from build123d import *

# Parameters (mm, degrees)
SKETCH1_W                                            = 152
SKETCH1_H                                            = 270
BOSS_EXTRUDE1_DEPTH                                  = 6
SKETCH2_R                                            = 35
CUT_EXTRUDE1_DEPTH                                   = 156.38661461
SKETCH5_R                                            = 6
SKETCH5_R_2                                          = 8.05
CUT_EXTRUDE2_DEPTH                                   = 5
SKETCH6_W                                            = 45
SKETCH6_H                                            = 70
CUT_EXTRUDE3_DEPTH                                   = 156.38661461
SKETCH7_W                                            = 45
SKETCH7_H                                            = 90
CUT_EXTRUDE4_DEPTH                                   = 156.38661461
SKETCH8_R                                            = 7.5
CUT_EXTRUDE5_DEPTH                                   = 2
SKETCH9_W                                            = 45
SKETCH9_H                                            = 65
CUT_EXTRUDE6_DEPTH                                   = 156.38661461
FILLET1_R                                            = 5
HOLE_SIZE_PER_SOCKET_HEAD_CAP_SCREW_TYPE_D           = 6.6
HOLE_SIZE_PER_SOCKET_HEAD_CAP_SCREW_TYPE_CBORE_D     = 11
HOLE_SIZE_PER_SOCKET_HEAD_CAP_SCREW_TYPE_CBORE_DEPTH = 6
HOLE_WIZARD_2_D                                      = 4.5
HOLE_WIZARD_2_CBORE_D                                = 8
HOLE_WIZARD_2_CBORE_DEPTH                            = 4
M8_CLEARANCE_HOLE1_D                                 = 8.4
CHAMFER1_SIZE                                        = 0.5


with BuildPart() as part:
    # Sketch1 → Boss-Extrude1 (new, symmetric)
    with BuildSketch(Plane(origin=(0, 0, 0), x_dir=(1, 0, 0), z_dir=(0, 1, 0))):
        Rectangle(SKETCH1_W, SKETCH1_H)
    extrude(amount=BOSS_EXTRUDE1_DEPTH, both=True)

    # Sketch2 → Cut-Extrude1 (cut, through all)
    with BuildSketch(Plane(origin=(0, 6, 0), x_dir=(1, 0, 0), z_dir=(0, 1, 0))):
        with Locations(Location((0, 0, 0), (0, 0, 270))):
            Circle(SKETCH2_R)
    extrude(amount=-CUT_EXTRUDE1_DEPTH, mode=Mode.SUBTRACT)

    # Sketch5 → Cut-Extrude2 (cut)
    with BuildSketch(Plane(origin=(0, 6, 0), x_dir=(1, 0, 0), z_dir=(0, 1, 0))):
        with Locations(Location((62.5, 62, 0), (0, 0, 270))):
            Circle(SKETCH5_R)
        with Locations(Location((-62.5, -62, 0), (0, 0, 270))):
            Circle(SKETCH5_R)
        with Locations(Location((62.5, 26, 0), (0, 0, 270))):
            Circle(SKETCH5_R_2)
        with Locations(Location((-62.5, 26, 0), (0, 0, 90))):
            Circle(SKETCH5_R_2)
        with Locations(Location((-62.5, -26, 0), (0, 0, 270))):
            Circle(SKETCH5_R_2)
        with Locations(Location((62.5, -26, 0), (0, 0, 90))):
            Circle(SKETCH5_R_2)
    extrude(amount=-CUT_EXTRUDE2_DEPTH, mode=Mode.SUBTRACT)

    # Sketch6 → Cut-Extrude3 (cut, through all)
    with BuildSketch(Plane(origin=(0, 6, 0), x_dir=(1, 0, 0), z_dir=(0, 1, 0))):
        Rectangle(SKETCH6_W, SKETCH6_H)
    extrude(amount=-CUT_EXTRUDE3_DEPTH, mode=Mode.SUBTRACT)

    # Sketch7 → Cut-Extrude4 (cut, through all)
    with BuildSketch(Plane(origin=(0, 6, 0), x_dir=(1, 0, 0), z_dir=(0, 1, 0))):
        with Locations((-53.5, 90)):
            Rectangle(SKETCH7_W, SKETCH7_H)
        with Locations((53.5, -90)):
            Rectangle(SKETCH7_W, SKETCH7_H)
    extrude(amount=-CUT_EXTRUDE4_DEPTH, mode=Mode.SUBTRACT)

    # Sketch8 → Cut-Extrude5 (cut)
    with BuildSketch(Plane.XZ.offset(6)):
        with Locations(Location((-20, 125, 0), (0, 0, 270))):
            Circle(SKETCH8_R)
        with Locations(Location((20, 125, 0), (0, 0, 90))):
            Circle(SKETCH8_R)
        with Locations(Location((20, -125, 0), (0, 0, 270))):
            Circle(SKETCH8_R)
        with Locations(Location((-20, -125, 0), (0, 0, 90))):
            Circle(SKETCH8_R)
    extrude(amount=-CUT_EXTRUDE5_DEPTH, mode=Mode.SUBTRACT)

    # Sketch9 → Cut-Extrude6 (cut, through all)
    with BuildSketch(Plane.XZ.offset(6)):
        with Locations((-53.5, 102.5)):
            Rectangle(SKETCH9_W, SKETCH9_H)
        with Locations((53.5, -102.5)):
            Rectangle(SKETCH9_W, SKETCH9_H)
    extrude(amount=-CUT_EXTRUDE6_DEPTH, mode=Mode.SUBTRACT)

    # Fillet1
    fillet1_edges = [part.edges().sort_by_distance(p)[0] for p in [
        (-31, 0, 70),
        (31, 0, -70),
        (22.5, 0, -35),
        (22.5, 0, 35),
        (-22.5, 0, 35),
        (-22.5, 0, -35),
        (-31, 0, -45),
        (31, 0, 45),
    ]]
    fillet(fillet1_edges, radius=FILLET1_R)

    # Hole size per socket head cap screw type 2 (through all)
    with Locations(Plane(origin=(0, 6, 0), x_dir=(1, 0, 0), z_dir=(0, 1, 0))):
        with Locations((-20, 125), (20, 125), (-20, -125), (20, -125)):
            CounterBoreHole(HOLE_SIZE_PER_SOCKET_HEAD_CAP_SCREW_TYPE_D / 2, HOLE_SIZE_PER_SOCKET_HEAD_CAP_SCREW_TYPE_CBORE_D / 2, HOLE_SIZE_PER_SOCKET_HEAD_CAP_SCREW_TYPE_CBORE_DEPTH)

    # 打孔尺寸(%根据)内六角圆柱头螺钉的类型2 (through all)
    with Locations(Plane(origin=(0, -6, 0), x_dir=(-1, 0, 0), z_dir=(0, -1, 0))):
        with Locations((62.5, -62), (-62.5, 62)):
            CounterBoreHole(HOLE_WIZARD_2_D / 2, HOLE_WIZARD_2_CBORE_D / 2, HOLE_WIZARD_2_CBORE_DEPTH)

    # M8 Clearance Hole1 (through all)
    with Locations(Plane(origin=(0, -6, 0), x_dir=(-1, 0, 0), z_dir=(0, -1, 0))):
        with Locations((62.5, -26), (62.5, 26), (-62.5, -26), (-62.5, 26)):
            Hole(M8_CLEARANCE_HOLE1_D / 2)

    # Chamfer1
    chamfer1_edges = [part.edges().sort_by_distance(p)[0] for p in [
        (-76, 0, 70),
        (-31, 0, 135),
        (76, 0, -70),
        (31, 0, -135),
        (-76, 0, -45),
        (-31, 0, -135),
        (76, 0, 45),
        (31, 0, 135),
    ]]
    chamfer(chamfer1_edges, length=CHAMFER1_SIZE)


solid = part.part
Geometry: final body of the model. Coordinates: model frame, mm. A direction names the side the tool comes from. Give positions to 0.01 mm unless a question says otherwise; leave off trailing zeros. Write each loop counter-clockwise with the first axis right and the second up, starting at its lowest first coordinate (ties: lowest second). Pieces come first, ordered by that corner, then holes.
(1) Cut plane A-A, the plane z = -125. Return loops of the section in (x, y), then the cut area to 3 significant figures.
(2) Ray query, line 1 (X direction, y = -5.25, z = 125); line 2 (X direction, y = 3, z = 124.5); line 3 (Z direction, x = -62.5, y = -4.85). Return the intervals inside material, ascending.
(3) Access query for faces 1 (the flat face through (0, 0, 35)), 2 (the cylindrical face through (19.284, 3.042, 119.547)), 3 (the flat face through (-31, 0, -92)), 4 (the flat face through (55, 0, -70)), 5 (the cylindrical face through (22.253, -5.014, -132.154)). Directions: +Z, -Z, +X, -X, +Y, -Y. A direction counts if a zero-diameter tool reaches every point of the face in a straight line with its end or side. Return the directions, or none.
(4) Cut plane C-C, the plane y = 3.75. Give the number of separate pieces and of enclosed holes in the cut face, then the cut area to 3 significant figures.
(5) Cut plane B-B, the plane z = -6.5. Return loops of the section in (x, y).
(6) Cut plane D-D, the plane x = -48. Return loops of the section in (y, z).
(7) First-contact query: P1, Ø10.5, axis at x = -20, z = 125, coming from the -Y side; P2, Ø1, axis at x = -44, y = 1.5, coming from the -Z side; P3, Ø1.5, axis at x = -33, y = -4, coming from the -Z side. Flat tips, straight axial feed; report the tip coordinate or a pass-through.
(8) Mould query, pull axis Z, two halves, no side actions, for faces 6 (the flat face through (76, 0, -12)), 7 (the flat face through (0, 0, -135)), 8 (the flat face through (55, 0, 45)), 9 (the flat face through (-64, -2, 64)). Classes: released by +Z, released by -Z, zero draft, split by the parting line, or undercut.
Values follow:
1. outline: (-31, -6) - (-27.5, -6) - (-27.5, -4) - (-23.3, -4) - (-23.3, 0) - (-25.5, 0) - (-25.5, 6) - (-31, 6) - close; (-16.7, -4) - (-12.5, -4) - (-12.5, -6) - (12.5, -6) - (12.5, -4) - (16.7, -4) - (16.7, 0) - (14.5, 0) - (14.5, 6) - (-14.5, 6) - (-14.5, 0) - (-16.7, 0) - close; (23.3, -4) - (27.5, -4) - (27.5, -6) - (31, -6) - (31, 6) - (25.5, 6) - (25.5, 0) - (23.3, 0) - close
1. area: 499 mm2
2. line 1: x = -31 to -27.5, -12.5 to 12.5, 27.5 to 31
2. line 2: x = -31 to -25.48, -14.52 to 14.52, 25.48 to 31
2. line 3: z = -45 to -30.2, -21.8 to 21.8, 30.2 to 58, 66 to 70
3. face 1: +Y, -Y
3. face 2: +Y
3. face 3: -Z, -X, +Y, -Y
3. face 4: -Z, +X, +Y, -Y
3. face 5: -Y
4. separate pieces: 1
4. enclosed holes: 11
4. area: 21,600 mm2
5. outline: (-76, -6) - (-34.39, -6) - (-34.39, 6) - (-76, 6) - close; (34.39, -6) - (76, -6) - (76, 6) - (34.39, 6) - close
6. outline: (-6, -45) - (6, -45) - (6, 70) - (-6, 70) - close
7. P1: stops at y = -4
7. P2: stops at z = -45
7. P3: stops at z = -46.69
8. face 6: zero draft
8. face 7: released by -Z
8. face 8: released by +Z
8. face 9: undercut
